The drawing under review shows one solid part. Ordinate dimensions are in mm from its lowest x, y, z. A direction names the side the tool comes from. Coordinates: 2 decimals unless noted, no trailing zeros. Order: outer loops, then holes, each group sorted by start corner. A loop starts at its lowest first (then second) coordinate and runs counter-clockwise, first axis right, second up. Notation, with made-up numbers: (33, 46.25) -> (76, 46.25) arc R5 ccw to (76, 55.25) -> close; hole circle Ø8 at (63, 27). An arc over 180 degrees is marked (long way). Use a Markdown table: item, result. Add a question column.
Q1. Machinability: for the marked faces 4 and 5, which of the approach directions +Z, -Z, +X, -X, +Y, -Y give a long, thin tool a straight path to every point of the face, cutting with its end or side? Answer none if there is none.
Q2. Wall thickness on probe 1 along Y at (x, z) = (15, 25); probe 2 along Y at (x, z) = (1.5, 15.25); probe 3 along Z at (x, y) = (11.75, 18.5) (1 decimal): over which ranges is each line inside the solid? List them lowest first.
Q3. Add section D-D (y = 11.75). State the section outline as (x, z) points.
Q4. The part is to be moulded in two halves that separate along Y. For the marked faces 1, 2 and 3, say which applies: pulls with the +Y half, pulls with the -Y half, needs draft (parallel to the pull), parting line crosses it, or undercut.
Q5. Add section A-A (z = 15). Count the separate pieces of the cut face and the enclosed holes in it, then the cut area to 3 significant figures.
Q6. Insertion check: pin 1 (5 mm diameter, centred on y = 9.5, z = 10, fed in from -X); pin 2 (2 mm diameter, centred on y = 13.5, z = 15.5, fed in from +X); pin 3 (4 mm diameter, centred on x = 15, y = 15, fed in from +Z); pin 4 (5 mm diameter, centred on x = 15, z = 15, fed in from -Y). Each pin has a flat end and moves straight along its axis. Give the tip position at first contact, or say it passes through.
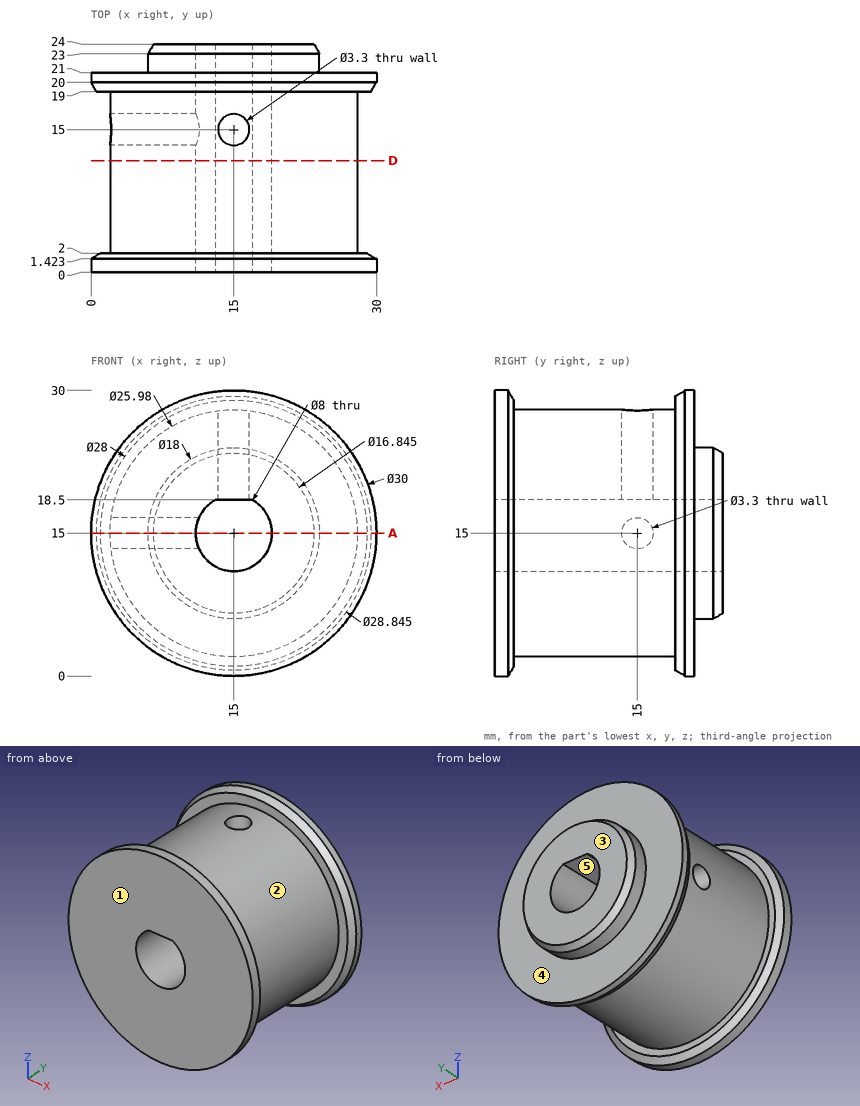
Established:
| question | item | result |
|---|---|---|
| 1 | face 4 | +Y |
| 1 | face 5 | +Y, -Y |
| 2 | probe 1 | 0 to 13.35, 16.65 to 21 |
| 2 | probe 2 | 0 to 2, 19 to 21 |
| 2 | probe 3 | 2.4 to 12.7, 17.3 to 27.6 |
| 3 | outline | circle Ø25.98 at (15, 15); hole (13.06, 18.5) arc R4 ccw (long way) to (16.94, 18.5) -> close |
| 4 | face 1 | pulls with the -Y half |
| 4 | face 2 | undercut |
| 4 | face 3 | pulls with the +Y half |
| 5 | separate pieces | 3 |
| 5 | enclosed holes | 0 |
| 5 | area | 392 mm^2 |
| 6 | pin 1 | x = 2.25 |
| 6 | pin 2 | x = 27.99 |
| 6 | pin 3 | z = 27.99 |
| 6 | pin 4 | through |
